For this review, take the finished solid that the model builds, in its own axes (mm). A direction names the side the tool comes from. Coordinates: 2 decimals unless noted, no trailing zeros. Order: outer loops, then holes, each group sorted by start corner. A loop starts at its lowest first (then second) coordinate and runs counter-clockwise, first axis right, second up. Notation, with made-up numbers: (-16, 88.25) - (32, 88.25) arc R19 ccw to (32, 92.25) - close; hole circle Ø3 at (7, 76.25). An arc over 180 degrees is marked (long way). One line per item, written item: value. Start each with the question number.
(1) Consider section C-C on y = -1. Write out the cut boundary in (x, z), then the cut area to 3 significant figures.
(2) Consider section A-A on z = 0. Write out the cut boundary in (x, y), then the cut area to 3 significant figures.
(3) Consider section D-D on x = 22. Write out the cut boundary in (y, z).
(4) For faces 4 (the flat face through (6, 55, 0)), 5 (the flat face through (-20, 37.5, 6)), 6 (the flat face through (0, -50, 0)), list the 3-axis set-ups (+Z, -Z, +X, -X, +Y, -Y) from which the entire face can be reached by the end or side of a thin tool; tool diameter is ignored.
(5) To check wall thickness, follow line 1 along Y through (x, z) = (14, 18.5); line 2 along X through (y, z) = (52.5, -22); line 3 along X through (y, z) = (53.5, -26.5). State the ranges of each line that lie inside material, in increasing order.
(6) Mouldability with a two-part tool opening along X and no side actions: class faces 1 (the cylindrical face through (-11.49, 50.175, 27.712)), 2 (the flat face through (16, 62.5, 0)), 3 (the flat face through (-6, 55, 0)) as released by +X, released by -X, zero draft, split by the parting line, or undercut.
(7) Clearance check with flat-ended pins moving along their axes: pin 1 (2 mm diameter, centred on y = -23, z = 6, fed in from +X); pin 2 (4 mm diameter, centred on y = -5, z = 19, fed in from -X); pin 3 (6 mm diameter, centred on x = 19.5, z = 15.5, fed in from -Y). State where each tip first meets the part, or that it passes through.
(8) Consider section B-B on x = 0. Write out the cut boundary in (y, z).
```python
from build123d import *

# Parameters (mm, degrees)
SKETCH_1_R          = 20
EXTRUDE_1_DEPTH     = 50
SKETCH_2_R          = 30
EXTRUDE_2_DEPTH     = 12.5
CHAMFER_1_SIZE      = 2
SKETCH_3_W          = 12
SKETCH_3_H          = 77.498414616
CUT_EXTRUDE_1_DEPTH = 15


with BuildPart() as part:
    # 草图1 → 凸台-拉伸1 (new, symmetric)
    with BuildSketch(Plane(origin=(0, 0, 0), x_dir=(1, 0, 0), z_dir=(0, 1, 0))):
        with Locations(Location((0, 0, 0), (0, 0, 270))):
            Circle(SKETCH_1_R)
    extrude(amount=EXTRUDE_1_DEPTH, both=True)

    # 草图2 → 凸台-拉伸2 (add, symmetric)
    with BuildSketch(Plane(origin=(0, 50, 0), x_dir=(1, 0, 0), z_dir=(0, 1, 0))):
        with Locations(Location((0, 0, 0), (0, 0, 270))):
            Circle(SKETCH_2_R)
    extrude(amount=EXTRUDE_2_DEPTH, both=True)

    # 倒角1
    chamfer_1_edges = [part.edges().sort_by_distance(p)[0] for p in [
        (0, -50, -20),
    ]]
    chamfer(chamfer_1_edges, length=CHAMFER_1_SIZE)

    # 草图3 → 切除-拉伸1 (cut)
    with BuildSketch(Plane(origin=(0, 62.5, 0), x_dir=(1, 0, 0), z_dir=(0, 1, 0))):
        Rectangle(SKETCH_3_W, SKETCH_3_H)
    extrude(amount=-CUT_EXTRUDE_1_DEPTH, mode=Mode.SUBTRACT)


solid = part.part
```
Geometry check:
1. outline: circle Ø40 at (0, 0)
1. area: 1,260 mm^2
2. outline: (-30, 37.5) - (-20, 37.5) - (-20, -48) - (-18, -50) - (18, -50) - (20, -48) - (20, 37.5) - (30, 37.5) - (30, 62.5) - (6, 62.5) - (6, 47.5) - (-6, 47.5) - (-6, 62.5) - (-30, 62.5) - close
2. area: 4,820 mm^2
3. outline: (37.5, -20.4) - (62.5, -20.4) - (62.5, 20.4) - (37.5, 20.4) - close
4. face 4: +Z, -Z, +Y
4. face 5: -Y
4. face 6: +Z, -Z, +X, -X, -Y
5. line 1: y = 37.5 to 62.5
5. line 2: x = -20.4 to -6, 6 to 20.4
5. line 3: x = -14.06 to -6, 6 to 14.06
6. face 1: split by the parting line
6. face 2: zero draft
6. face 3: undercut
7. pin 1: stops at x = 19.36
7. pin 2: stops at x = -10.54
7. pin 3: stops at y = 37.5
8. outline: (-50, -18) - (-48, -20) - (37.5, -20) - (37.5, -30) - (47.5, -30) - (47.5, 30) - (37.5, 30) - (37.5, 20) - (-48, 20) - (-50, 18) - close
